```python
from build123d import *

# Parameters (mm, degrees)
SKETCH1_R                = 17.5
BOSS_EXTRUDE1_DEPTH      = 30
SKETCH2_R                = 4
BOSS_EXTRUDE2_DEPTH      = 2
CHAMFER1_SIZE            = 1
SKETCH4_R                = 2
BOSS_EXTRUDE3_DEPTH      = 12
SKETCH5_R                = 1.5
CUT_EXTRUDE1_DEPTH       = 12
CUT_EXTRUDE2_DEPTH       = 39.890872965
CUT_EXTRUDE2_DEPTH_BACK  = 39.890872965
SKETCH6_W                = 34.294260261
SKETCH6_H                = 28
CUT_EXTRUDE3_DEPTH       = 39.890872965
CUT_EXTRUDE3_DEPTH_BACK  = 39.890872965
SKETCH7_W                = 3
SKETCH7_H                = 23
CUT_EXTRUDE4_DEPTH       = 39.890872965
CUT_EXTRUDE4_DEPTH_BACK  = 39.890872965
SKETCH8_W                = 1.5
SKETCH8_H                = 5
CUT_EXTRUDE5_DEPTH       = 48.908767465
CUT_EXTRUDE5_DEPTH_BACK  = 48.908767465
SKETCH9_W                = 8.124038405
SKETCH9_H                = 23
CUT_EXTRUDE6_DEPTH       = 51.482670294
CUT_EXTRUDE6_DEPTH_BACK  = 0.5
SKETCH10_R               = 0.641252557
SKETCH11_R               = 17.5
BOSS_EXTRUDE4_DEPTH      = 5
CUT_EXTRUDE8_DEPTH       = 4
CUT_EXTRUDE9_DEPTH       = 39.890872965
CUT_EXTRUDE9_DEPTH_BACK  = 39.890872965
SKETCH13_W               = 19.268240878
SKETCH13_H               = 2
SKETCH14_R               = 2
CUT_EXTRUDE10_DEPTH      = 6
CUT_EXTRUDE11_DEPTH      = 39.890872965
CUT_EXTRUDE11_DEPTH_BACK = 39.890872965
SKETCH16_W               = 3.25
SKETCH16_H               = 3
CUT_EXTRUDE12_DEPTH      = 36.178118199
CUT_EXTRUDE13_START      = -17
SKETCH18_R               = 17.5
CUT_EXTRUDE13_DEPTH      = 17
BOSS_EXTRUDE5_DEPTH      = 3
BOSS_EXTRUDE6_DEPTH      = 13
CUT_EXTRUDE14_DEPTH      = 46.348649373
CUT_EXTRUDE14_DEPTH_BACK = 46.348649373
SKETCH21_R               = 1.5
SKETCH22_R               = 1
BOSS_EXTRUDE7_DEPTH      = 5
CUT_EXTRUDE15_DEPTH      = 5


with BuildPart() as part:
    # Sketch1 → Boss-Extrude1 (new body)
    with BuildSketch(Plane(origin=(0, 0, 0), x_dir=(1, 0, 0), z_dir=(0, 1, 0))):
        with Locations(Location((0, 0, 0), (0, 0, 270))):
            Circle(SKETCH1_R)
    extrude(amount=BOSS_EXTRUDE1_DEPTH)

    # Sketch2 → Boss-Extrude2 (add)
    with BuildSketch(Plane.XZ):
        with Locations(Location((0, 0, 0), (0, 0, 270))):
            Circle(SKETCH2_R)
    extrude(amount=BOSS_EXTRUDE2_DEPTH)

    # Chamfer1
    chamfer1_edges = [part.edges().sort_by_distance(p)[0] for p in [
        (0, 0, 4),
    ]]
    chamfer(chamfer1_edges, length=CHAMFER1_SIZE)

    # Sketch4 → Boss-Extrude3 (add)
    with BuildSketch(Plane.XZ.offset(2)):
        with Locations(Location((0, 0, 0), (0, 0, 270))):
            Circle(SKETCH4_R)
    extrude(amount=BOSS_EXTRUDE3_DEPTH)

    # Sketch5 → Cut-Extrude1 (cut)
    with BuildSketch(Plane.XZ.offset(14)):
        with Locations(Location((0, 0, 0), (0, 0, 270))):
            Circle(SKETCH5_R)
    extrude(amount=-CUT_EXTRUDE1_DEPTH, mode=Mode.SUBTRACT)

    # Sketch6 → Cut-Extrude2 (cut, two sides: drawn at the far end of the back side and taken through both)
    with BuildSketch(Plane(origin=(0, 0, 0), x_dir=(0, 0, -1), z_dir=(1, 0, 0)).offset(-CUT_EXTRUDE2_DEPTH_BACK)):
        with Locations((4.647130131, 16)):
            Rectangle(SKETCH6_W, SKETCH6_H)
    extrude(amount=CUT_EXTRUDE2_DEPTH + CUT_EXTRUDE2_DEPTH_BACK, mode=Mode.SUBTRACT)

    # Sketch7 → Cut-Extrude3 (cut, two sides: drawn at the far end of the back side and taken through both)
    with BuildSketch(Plane(origin=(0, 0, 0), x_dir=(0, 0, -1), z_dir=(1, 0, 0)).offset(-CUT_EXTRUDE3_DEPTH_BACK)):
        with Locations((-14, 18.5)):
            Rectangle(SKETCH7_W, SKETCH7_H)
    extrude(amount=CUT_EXTRUDE3_DEPTH + CUT_EXTRUDE3_DEPTH_BACK, mode=Mode.SUBTRACT)

    # Sketch8 → Cut-Extrude4 (cut, two sides: drawn at the far end of the back side and taken through both)
    with BuildSketch(Plane(origin=(0, 0, 0), x_dir=(0, 0, -1), z_dir=(1, 0, 0)).offset(-CUT_EXTRUDE4_DEPTH_BACK)):
        with Locations((-13.25, 4.5)):
            Rectangle(SKETCH8_W, SKETCH8_H)
    extrude(amount=CUT_EXTRUDE4_DEPTH + CUT_EXTRUDE4_DEPTH_BACK, mode=Mode.SUBTRACT)

    # Sketch9 → Cut-Extrude5 (cut, two sides: drawn at the far end of the back side and taken through both)
    with BuildSketch(Plane(origin=(0, 0, 15.5), x_dir=(-1, 0, 0), z_dir=(0, 0, -1)).offset(-CUT_EXTRUDE5_DEPTH_BACK)):
        with Locations((-4.062019203, 18.5)):
            Rectangle(SKETCH9_W, SKETCH9_H)
    extrude(amount=CUT_EXTRUDE5_DEPTH + CUT_EXTRUDE5_DEPTH_BACK, mode=Mode.SUBTRACT)

    # Sketch10 → Cut-Extrude6 (cut, two sides: drawn at the far end of the back side and taken through both)
    with BuildSketch(Plane(origin=(0, 30, 0), x_dir=(1, 0, 0), z_dir=(0, 1, 0)).offset(-CUT_EXTRUDE6_DEPTH_BACK)):
        with Locations(Location((-1.034007802, -16.523277445, 0), (0, 0, 270))):
            Circle(SKETCH10_R)
    extrude(amount=CUT_EXTRUDE6_DEPTH + CUT_EXTRUDE6_DEPTH_BACK, mode=Mode.SUBTRACT)

    # Sketch11 → Boss-Extrude4 (add)
    with BuildSketch(Plane(origin=(0, 2, 0), x_dir=(1, 0, 0), z_dir=(0, 1, 0))):
        with Locations(Location((0, 0, 0), (0, 0, 270))):
            Circle(SKETCH11_R)
    extrude(amount=BOSS_EXTRUDE4_DEPTH)

    # Sketch12 → Cut-Extrude8 (cut)
    with BuildSketch(Plane(origin=(0, 7, 0), x_dir=(1, 0, 0), z_dir=(0, 1, 0))):
        with BuildLine():
            Line((-17.5, 0), (-3, 0))
            ThreePointArc((-3, 0), (0, 3), (3, 0))
            Line((3, 0), (11, 0))
            ThreePointArc((11, 0), (12.5, 1.5), (14, 0))
            Line((14, 0), (18.571441089, 0))
            Line((18.571441089, 0), (18.571441089, 21.35501059))
            Line((18.571441089, 21.35501059), (-17.5, 21.35501059))
            Line((-17.5, 21.35501059), (-17.5, 0))
        make_face()
    extrude(amount=-CUT_EXTRUDE8_DEPTH, mode=Mode.SUBTRACT)

    # Sketch13 → Cut-Extrude9 (cut, two sides: drawn at the far end of the back side and taken through both)
    with BuildSketch(Plane(origin=(0, 0, 0), x_dir=(0, 0, -1), z_dir=(1, 0, 0)).offset(-CUT_EXTRUDE9_DEPTH_BACK)):
        with Locations((-4.288358488, 6)):
            Rectangle(SKETCH13_W, SKETCH13_H)
    extrude(amount=CUT_EXTRUDE9_DEPTH + CUT_EXTRUDE9_DEPTH_BACK, mode=Mode.SUBTRACT)

    # Sketch14 → Cut-Extrude10 (cut)
    with BuildSketch(Plane(origin=(0, 5, 0), x_dir=(1, 0, 0), z_dir=(0, 1, 0))):
        with Locations(Location((0, 0, 0), (0, 0, 90))):
            Circle(SKETCH14_R)
    extrude(amount=-CUT_EXTRUDE10_DEPTH, mode=Mode.SUBTRACT)

    # Sketch16 → Cut-Extrude11 (cut, two sides: drawn at the far end of the back side and taken through both)
    with BuildSketch(Plane(origin=(0, 0, 0), x_dir=(0, 0, -1), z_dir=(1, 0, 0)).offset(-CUT_EXTRUDE11_DEPTH_BACK)):
        with Locations((15.875, 1.5)):
            Rectangle(SKETCH16_W, SKETCH16_H)
    extrude(amount=CUT_EXTRUDE11_DEPTH + CUT_EXTRUDE11_DEPTH_BACK, mode=Mode.SUBTRACT)

    # Sketch17 → Cut-Extrude12 (cut, through all)
    with BuildSketch(Plane(origin=(0, 5, 0), x_dir=(1, 0, 0), z_dir=(0, 1, 0))):
        with BuildLine():
            ThreePointArc((9.545941546, -9.545941546), (12.472373689, -5.166226337), (13.5, 0))
            ThreePointArc((13.5, 0), (12.5, 1), (11.5, 0))
            ThreePointArc((11.5, 0), (10.624614624, -4.400859472), (8.131727984, -8.131727984))
            ThreePointArc((8.131727984, -8.131727984), (8.131727984, -9.545941546), (9.545941546, -9.545941546))
        make_face()
    extrude(amount=-CUT_EXTRUDE12_DEPTH, mode=Mode.SUBTRACT)

    # Sketch18 → Cut-Extrude13 (cut)
    with BuildSketch(Plane(origin=(0, 3, 0), x_dir=(1, 0, 0), z_dir=(0, 1, 0)).offset(CUT_EXTRUDE13_START)):
        Circle(SKETCH18_R)
    extrude(amount=CUT_EXTRUDE13_DEPTH, mode=Mode.SUBTRACT)

    # Sketch19 → Boss-Extrude5 (add)
    with BuildSketch(Plane(origin=(0, 7, 0), x_dir=(1, 0, 0), z_dir=(0, 1, 0))):
        with BuildLine():
            Line((10.602574241, -13.922478927), (-10.602574241, -13.922478927))
            ThreePointArc((-10.602574241, -13.922478927), (-9.396470001, -14.763344862), (-8.124038405, -15.5))
            Line((-8.124038405, -15.5), (0, -15.5))
            Line((0, -15.5), (0, -17.5))
            ThreePointArc((0, -17.5), (5.594936049, -16.581516535), (10.602574241, -13.922478927))
        make_face()
    extrude(amount=BOSS_EXTRUDE5_DEPTH)

    # Sketch20 → Boss-Extrude6 (add)
    with BuildSketch(Plane(origin=(0, 30, 0), x_dir=(1, 0, 0), z_dir=(0, 1, 0))):
        with BuildLine():
            Line((0, -17.5), (0, -15.5))
            Line((0, -15.5), (-8.124038405, -15.5))
            ThreePointArc((-8.124038405, -15.5), (-4.183300133, -16.992645468), (0, -17.5))
        make_face()
    extrude(amount=BOSS_EXTRUDE6_DEPTH)

    # Sketch21 → Cut-Extrude14 (cut, two sides: drawn at the far end of the back side and taken through both)
    with BuildSketch(Plane(origin=(0, 5, 0), x_dir=(1, 0, 0), z_dir=(0, 1, 0)).offset(-CUT_EXTRUDE14_DEPTH_BACK)):
        with Locations((-12.5, 0)):
            Circle(SKETCH21_R)
    extrude(amount=CUT_EXTRUDE14_DEPTH + CUT_EXTRUDE14_DEPTH_BACK, mode=Mode.SUBTRACT)

    # Sketch22 → Boss-Extrude7 (add)
    with BuildSketch(Plane(origin=(0, 5, 0), x_dir=(1, 0, 0), z_dir=(0, 1, 0))):
        with Locations(Location((-10.580817493, -6.655546647, 0), (0, 0, 90))):
            Circle(SKETCH22_R)
    extrude(amount=BOSS_EXTRUDE7_DEPTH)

    # Sketch23 → Cut-Extrude15 (cut)
    with BuildSketch(Plane(origin=(0, 5, 0), x_dir=(1, 0, 0), z_dir=(0, 1, 0))):
        with BuildLine():
            Line((-14, 0), (-3, 0))
            ThreePointArc((-3, 0), (-8.5, -4.635701065), (-14, 0))
        make_face()
    extrude(amount=-CUT_EXTRUDE15_DEPTH, mode=Mode.SUBTRACT)


solid = part.part
```
Geometry: final body of the model. Coordinates: model frame, mm. A direction names the side the tool comes from. Coordinates: 2 decimals unless noted, no trailing zeros. Order: outer loops, then holes, each group sorted by start corner. A loop starts at its lowest first (then second) coordinate and runs counter-clockwise, first axis right, second up. Notation, with made-up numbers: (74.5, 15.25) -> (132.5, 15.25) arc R17 cw to (132.5, 32.25) -> close; hole circle Ø2 at (43, 40.5). An arc over 180 degrees is marked (long way). Write each question's results on one line, items separated by ' | '. Start each with the question number.
1) Cut plane C-C, the plane x = -13. Output: boundary loops of the cut face in (y, z).
2) Set-up query: faces 1 (the flat face through (-16, 4, 0)), 2 (the flat face through (-1, 30, 17)), 3 (the flat face through (0, 26, 17)). Return all of +Z, -Z, +X, -X, +Y, -Y with unobstructed straight access to the full face (end or side cutting, diameter ignored); none if empty.
3) First-contact query: pin 1 (5 mm diameter, centred on x = 1, z = 7, fed in from +Y); pin 2 (1.1 mm diameter, centred on x = 4.5, z = 16, fed in from +Y); pin 3 (1.6 mm diameter, centred on x = -16, y = 4.5, fed in from -Z); pin 4 (2 mm diameter, centred on y = 19.5, z = 13.5, fed in from -X). Flat tips, straight axial feed; report the tip coordinate or a pass-through.
4) Mould query, pull axis X, two halves, no side actions, for faces 4 (the cylindrical face through (-11.26, 7.46, 7.39)), 5 (the flat face through (-3, 43, 16)), 6 (the cylindrical face through (-1.006, 29.746, 15.883)), 7 (the cylindrical face through (12.5, 4, -1.5)). Classes: released by +X, released by -X, zero draft, split by the parting line, or undercut.
5) Cut plane A-A, the plane x = 12.5. Output: boundary loops of the cut face in (y, z), and give its area (3 significant figures).
6) Cut plane B-B, the plane y = 39. Output: boundary loops of the cut face in (x, z), and give its area (3 significant figures).
7) Material intervals for line 1 along Y through (x, z) = (9, 1.5); line 2 along X through (y, z) = (8.5, 6.5); line 3 along X through (y, z) = (33, 15.75), sorted ascending.
Checks:
1) outline: (3, 2.36) -> (5, 2.36) -> (5, 11.72) -> (3, 11.72) -> close
2) face 1: -Z, -X, +Y, -Y | face 2: none | face 3: +Z, -Z, +X, +Y
3) pin 1: y = 5 | pin 2: y = 10 | pin 3: z = 0 | pin 4: through
4) face 4: split by the parting line | face 5: zero draft | face 6: undercut | face 7: undercut
5) outline: (3, -1.5) -> (5, -1.5) -> (5, -1) -> (3, -1) -> close; (3, 5.1) -> (5, 5.1) -> (5, 12.25) -> (3, 12.25) -> close | area: 15.3 mm^2
6) outline: (-8.12, 15.5) -> (0, 15.5) -> (0, 17.5) arc R17.5 ccw to start | area: 11.0 mm^2
7) line 1: 3 to 5 | line 2: -11.57 to -9.59 | line 3: -7.63 to 0
